```python
from build123d import *

# Parameters (mm, degrees)
CUT_EXTRUDE_1_DEPTH      = 3
CUT_EXTRUDE_1_DEPTH_BACK = 3
SKETCH_2_R               = 45
SCALE_1_SCALE            = 0.5


with BuildPart() as part:
    # 草图1 → 旋转1 (revolve)
    with BuildSketch(Plane.XY, mode=Mode.PRIVATE) as revolve_1_sk:
        Polygon((-3, 6), (-3, 4), (-2.3235, 3.3235), (2.3235, 3.3235), (3, 4), (3, 6), (0, 13.242640687), align=None)
    revolve(revolve_1_sk.sketch.rotate(Axis((3, 0, 0), (-1, 0, 0)), 180), axis=Axis((3, 0, 0), (-1, 0, 0)))

    # 草图2 → 切除-拉伸1 (cut, two sides: drawn at the far end of the back side and taken through both)
    with BuildSketch(Plane(origin=(0, 0, 0), x_dir=(0, 0, -1), z_dir=(1, 0, 0)).offset(-CUT_EXTRUDE_1_DEPTH_BACK)):
        Circle(SKETCH_2_R)
        Polygon((-6, -3.464101615), (0, -6.92820323), (6, -3.464101615), (6, 3.464101615), (0, 6.92820323), (-6, 3.464101615), align=None, mode=Mode.SUBTRACT)
    extrude(amount=CUT_EXTRUDE_1_DEPTH + CUT_EXTRUDE_1_DEPTH_BACK, mode=Mode.SUBTRACT)


with BuildPart() as part_1:
    # 缩放比例1: scaled about (0, 1e-09, 0)
    add(part.part.scale(SCALE_1_SCALE).moved(Location((0, 1e-09, 0))))


solid = part_1.part
```
The model under review builds one solid part; all positions refer to its coordinate system, in mm. Round coordinates to 2 decimals unless told otherwise and drop trailing zeros. Loops run counter-clockwise (first coordinate to the right, second up) from the corner with the lowest first, then second, coordinate; pieces in that order, holes last. Notation, with made-up numbers: M 66,-7.75 L 115,-7.75 A31 ccw 115,18.25 Z; hole C -37.5,28 d9. An arc over 180 degrees is marked long. Put each result on its own line as item: value.
Q1. Mouldability with a two-part tool opening along Z and no side actions: class faces 1 (the flat face through (0, 2.6, -1.5)), 2 (the cylindrical face through (0.016, -0.767, -1.474)), 3 (the conical face through (-1.433, 1.574, 2.742)) as released by +Z, released by -Z, zero draft, split by the parting line, or undercut.
Result set:
face 1: released by -Z
face 2: undercut
face 3: released by +Z
Q2. Consider section A-A, the plane x = 0.5. Give the boundary of the cut face in (y, z).
Result set:
outline: M -3.46,0 L -1.73,-3 L 1.73,-3 L 3.46,0 L 1.73,3 L -1.73,3 Z; hole C 0,0 d3.32
Q3. To check wall thickness, follow L1, parallel to Y at x = 0.3, z = 1.25; L2, parallel to Y at x = -0.35, z = -2; L3, parallel to Y at x = -0.3, z = -0.5. State the ranges of each line that lie inside material, in increasing order.
Result set:
L1: y = -2.74 to -1.09, 1.09 to 2.74
L2: y = -2.31 to 2.31
L3: y = -3.18 to -1.58, 1.58 to 3.18
Q4. For pin 1 (1.5 mm diameter, centred on x = -1, z = -2, fed in from -Y); pin 2 (1 mm diameter, centred on x = 1, z = -1.5, fed in from +Y), all flat-tipped, find the tip position at first contact; note any pin that passes through.
Result set:
pin 1: stops at y = -2.74
pin 2: stops at y = 2.89
